Part model, mm, in its own coordinate system. A direction names the side the tool comes from. Coordinates: 2 decimals unless noted, no trailing zeros. Loops run counter-clockwise (first coordinate to the right, second up) from the corner with the lowest first, then second, coordinate; pieces in that order, holes last. Notation, with made-up numbers: (18.25, 86.5) - (36.25, 86.5) arc R22 cw to (36.25, 108.5) - close; hole circle Ø6 at (35, 8). An arc over 180 degrees is marked (long way). Answer as CSV lines item,"result".
from build123d import *

# Parameters (mm, degrees)
EXTRUDE_1_DEPTH     = 5
CUT_EXTRUDE_1_REACH = 186.989
SKETCH_2_R          = 2.5
SKETCH_3_W          = 14
SKETCH_3_H          = 50
EXTRUDE_2_DEPTH     = 10
FILLET_1_R          = 5
CHAMFER_1_SIZE      = 2


with BuildPart() as part:
    # 草图1 → 凸台-拉伸1 (new, symmetric)
    with BuildSketch(Plane.XY):
        Polygon((0, 0), (-85, 0), (-85, 164), (-65, 164), (-65, 14), (85, 14), (85, 0), align=None)
    extrude(amount=EXTRUDE_1_DEPTH, both=True)

    # 草图2 → 切除-拉伸1 (cut, up to next)
    with BuildSketch(Plane.XY.offset(5), mode=Mode.PRIVATE) as cut_extrude_1_sk1:
        with Locations((-80, 159)):
            Circle(SKETCH_2_R)
    cut_extrude_1_tool1 = extrude(cut_extrude_1_sk1.sketch, amount=-CUT_EXTRUDE_1_REACH, mode=Mode.PRIVATE) & part.part
    # 草图2 → 切除-拉伸1 (cut, up to next)
    with BuildSketch(Plane.XY.offset(5), mode=Mode.PRIVATE) as cut_extrude_1_sk2:
        with Locations((-70, 159)):
            Circle(SKETCH_2_R)
    cut_extrude_1_tool2 = extrude(cut_extrude_1_sk2.sketch, amount=-CUT_EXTRUDE_1_REACH, mode=Mode.PRIVATE) & part.part
    add(cut_extrude_1_tool1.solids().sort_by_distance((-80, 159, 5))[0], mode=Mode.SUBTRACT)
    add(cut_extrude_1_tool2.solids().sort_by_distance((-70, 159, 5))[0], mode=Mode.SUBTRACT)

    # 草图3 → 凸台-拉伸2 (add)
    with BuildSketch(Plane.XY.offset(5)):
        with Locations((78, -25)):
            Rectangle(SKETCH_3_W, SKETCH_3_H)
    extrude(amount=-EXTRUDE_2_DEPTH)

    # 圆角1
    fillet_1_edges = [part.edges().sort_by_distance(p)[0] for p in [
        (-65, 14, 0),
        (71, 0, 0),
    ]]
    fillet(fillet_1_edges, radius=FILLET_1_R)

    # 倒角1
    chamfer_1_edges = [part.edges().sort_by_distance(p)[0] for p in [
        (-85, 0, 0),
        (85, 14, 0),
    ]]
    chamfer(chamfer_1_edges, length=CHAMFER_1_SIZE)


solid = part.part
Q1. Which spindle directions (+Z, -Z, +X, -X, +Y, -Y) get a long thin tool onto all of the face, cutting with end or side? Do faces 4 (the face through (-65, 93, 0)), 5 (the face through (85, -19, 0)), 6 (the face through (71, -28, 0)). Say none if no direction does.
Results:
face 4,"+Z, -Z, +X, +Y"
face 5,"+Z, -Z, +X, +Y, -Y"
face 6,"+Z, -Z, -X, -Y"
Q2. Flat gauge pins, fed straight in: pin 1 (3 mm diameter, centred on x = -64.5, z = -2.5, fed in from -Y); pin 2 (1 mm diameter, centred on y = 134.5, z = 2.5, fed in from +X); pin 3 (1.5 mm diameter, centred on x = -9.5, z = -2, fed in from +Y); pin 4 (8 mm diameter, centred on x = -70, y = 159, fed in from -Z). Where does each tip first touch, or does it go through?
Results:
pin 1,"stops at y = 0"
pin 2,"stops at x = -65"
pin 3,"stops at y = 14"
pin 4,"stops at z = -5"
Q3. Wall check: L1, parallel to X at y = 159, z = 1.75; L2, parallel to Y at x = -80, z = 1.5; L3, parallel to Y at x = -30.5, z = 4.25. Give the ranges that are in metal, low to high.
Results:
L1,"x = -85 to -82.5, -77.5 to -72.5, -67.5 to -65"
L2,"y = 0 to 156.5, 161.5 to 164"
L3,"y = 0 to 14"
Q4. Two-plate mould, pull along Y, no slides. Class faces 1 (the face through (78, -50, 0)), 2 (the face through (-85, 82, 0)), 3 (the face through (-80.33, 161.48, 0.07)): released by +Y, released by -Y, zero draft, split by the parting line, or undercut.
Results:
face 1,"released by -Y"
face 2,"zero draft"
face 3,"undercut"
Q5. Saw through at A-A (y = 159). Give the cut face in (x, z).
Results:
outline,"(-85, -5) - (-82.5, -5) - (-82.5, 5) - (-85, 5) - close; (-77.5, -5) - (-72.5, -5) - (-72.5, 5) - (-77.5, 5) - close; (-67.5, -5) - (-65, -5) - (-65, 5) - (-67.5, 5) - close"
Q6. Saw through at B-B (x = -80). Give the cut face in (y, z).
Results:
outline,"(0, -5) - (156.5, -5) - (156.5, 5) - (0, 5) - close; (161.5, -5) - (164, -5) - (164, 5) - (161.5, 5) - close"
Q7. Saw through at D-D (y = 81.5). Give the cut face in (x, z).
Results:
outline,"(-85, -5) - (-65, -5) - (-65, 5) - (-85, 5) - close"
Q8. Saw through at C-C (z = 1.5). Give the cut face in (x, y), then the cut area to 3 significant figures.
Results:
outline,"(-85, 2) - (-83, 0) - (66, 0) arc R5 cw to (71, -5) - (71, -50) - (85, -50) - (85, 12) - (83, 14) - (-60, 14) arc R5 cw to (-65, 19) - (-65, 164) - (-85, 164) - close; hole circle Ø5 at (-80, 159); hole circle Ø5 at (-70, 159)"
area,"6,050 mm^2"
